from build123d import *

# Parameters (mm, degrees)
EXTRUDE1_DEPTH                 = 6.35
F_9_16_0_5625_DIAMETER_HOLE1_D = 14.2875
F_3_8_0_375_DIAMETER_HOLE1_D   = 9.525


with BuildPart() as part:
    # Sketch1 → Extrude1 (new body)
    with BuildSketch(Plane.XY):
        with BuildLine():
            Line((0, 53.05662155), (0, 561.62337845))
            ThreePointArc((0, 561.62337845), (15.539924665, 599.140075335), (53.05662155, 614.68))
            Line((53.05662155, 614.68), (731.94337845, 614.68))
            ThreePointArc((731.94337845, 614.68), (769.460075335, 599.140075335), (785, 561.62337845))
            Line((785, 561.62337845), (785, 421.05662155))
            ThreePointArc((785, 421.05662155), (800.539924665, 383.539924665), (838.05662155, 368))
            Line((838.05662155, 368), (944.94337845, 368))
            ThreePointArc((944.94337845, 368), (982.460075335, 352.460075335), (998, 314.94337845))
            Line((998, 314.94337845), (998, 53.05662155))
            ThreePointArc((998, 53.05662155), (982.460075335, 15.539924665), (944.94337845, 0))
            Line((944.94337845, 0), (53.05662155, 0))
            ThreePointArc((53.05662155, 0), (15.539924665, 15.539924665), (0, 53.05662155))
        make_face()
        with BuildLine():
            Line((698.28, 104.14), (774.48, 104.14))
            ThreePointArc((774.48, 104.14), (783.460256121, 107.859743879), (787.18, 116.84))
            Line((787.18, 116.84), (787.18, 243.84))
            ThreePointArc((787.18, 243.84), (783.460256121, 252.820256121), (774.48, 256.54))
            Line((774.48, 256.54), (698.28, 256.54))
            ThreePointArc((698.28, 256.54), (689.299743879, 252.820256121), (685.58, 243.84))
            Line((685.58, 243.84), (685.58, 116.84))
            ThreePointArc((685.58, 116.84), (689.299743879, 107.859743879), (698.28, 104.14))
        make_face(mode=Mode.SUBTRACT)
    extrude(amount=EXTRUDE1_DEPTH)

    # 9/16 (0.5625) Diameter Hole1 (through all)
    with Locations(Plane.XY.offset(6.35)):
        with Locations((22.61, 309.62), (29.72, 512.82), (27.44, 106.42), (92.46, 20.57), (92.46, 593.59), (694.19, 593.59), (393.96, 593.59), (359.16, 20.57), (625.86, 20.57), (892.56, 20.57), (978.16, 96.77), (982.22, 309.62), (770.39, 388.87)):
            Hole(F_9_16_0_5625_DIAMETER_HOLE1_D / 2)

    # 3/8 (0.375) Diameter Hole1 (through all)
    with Locations(Plane.XY.offset(6.35)):
        with Locations((684.28, 264.92), (684.28, 96.77), (801.63, 96.77), (801.63, 264.92)):
            Hole(F_3_8_0_375_DIAMETER_HOLE1_D / 2)


solid = part.part
Design review of the part built by this model. Coordinates are the model's own, in mm. Give positions to 0.01 mm unless a question says otherwise; leave off trailing zeros. Order: outer loops, then holes, each group sorted by start corner. A loop starts at its lowest first (then second) coordinate and runs counter-clockwise, first axis right, second up. Notation, with made-up numbers: (-19, -27.75) - (13, -27.75) arc R30 ccw to (13, 7.25) - close; hole circle Ø5 at (14.25, 48). An arc over 180 degrees is marked (long way). Use CSV: the item, a comma, the result in double quotes. Start each with the question number.
Q1. For P1, Ø8.5, axis at x = 27.44, y = 106.42, coming from the -Z side; P2, Ø3, axis at x = 905.5, z = 2, coming from the +Y side, all flat-tipped, find the tip position at first contact; note any pin that passes through.
Q2. Take a section at C-C (y = 486.5). State the section outline as (x, z) points, and give its area (3 significant figures).
Q3. Take a section at A-A (y = 230.5). State the section outline as (x, z) points, and give its area (3 significant figures).
Q4. Take a section at B-B (z = 3). Count the separate pieces of the cut face and the enclosed holes in it, and give its area (3 significant figures).
Q5. For line 1 (Y direction, x = 801.63, z = 4.5); line 2 (X direction, y = 141, z = 1); line 3 (X direction, y = 593.59, z = 1.5), list the stretches that pass through material, from the lowest coordinate up.
Calculated:
1,P1,"passes through"
1,P2,"stops at y = 368"
2,outline,"(0, 0) - (785, 0) - (785, 6.35) - (0, 6.35) - close"
2,area,"4,980 mm²"
3,outline,"(0, 0) - (685.58, 0) - (685.58, 6.35) - (0, 6.35) - close; (787.18, 0) - (998, 0) - (998, 6.35) - (787.18, 6.35) - close"
3,area,"5,690 mm²"
4,separate pieces,"1"
4,enclosed holes,"18"
4,area,"541,000 mm²"
5,line 1,"y = 0 to 92.01, 101.53 to 260.16, 269.68 to 382.48"
5,line 2,"x = 0 to 685.58, 787.18 to 998"
5,line 3,"x = 10.71 to 85.32, 99.6 to 386.82, 401.1 to 687.05, 701.33 to 774.29"
